Work out the finished part from the listing and answer in its coordinate system (mm). Round coordinates to 2 decimals unless told otherwise and drop trailing zeros. Write each loop counter-clockwise with the first axis right and the second up, starting at its lowest first coordinate (ties: lowest second). Pieces come first, ordered by that corner, then holes. Notation, with made-up numbers: M -15,15 L 41,15 A26 ccw 41,34 Z; hole C -14.5,18 d5. An arc over 180 degrees is marked long. Answer in a Markdown table with one row per item.
```python
from build123d import *

# Parameters (mm, degrees)
SKETCH1_W                  = 80
SKETCH1_H                  = 105
BOSS_EXTRUDE1_DEPTH        = 3
SKETCH2_R                  = 2.75
SKETCH2_R_2                = 25.05
CUT_EXTRUDE1_DEPTH         = 133.037873355
F_4_5_4_5_DIAMETER_HOLE1_D = 4.5
CHAMFER1_SIZE              = 2
M4_TAPPED_HOLE1_D          = 3.3
M4_TAPPED_HOLE1_DEPTH      = 10.1
M4_TAPPED_HOLE1_TIP        = 0.991420021


with BuildPart() as part:
    # Sketch1 → Boss-Extrude1 (new body)
    with BuildSketch(Plane.XY):
        with Locations((40, 52.5)):
            Rectangle(SKETCH1_W, SKETCH1_H)
    extrude(amount=BOSS_EXTRUDE1_DEPTH)

    # Sketch2 → Cut-Extrude1 (cut, through all)
    with BuildSketch(Plane.XY.offset(3)):
        with Locations((7.5, 97.5)):
            Circle(SKETCH2_R)
        with Locations((72.5, 97.5)):
            Circle(SKETCH2_R)
        with Locations((72.5, 7.5)):
            Circle(SKETCH2_R)
        with Locations((7.5, 7.5)):
            Circle(SKETCH2_R)
        with Locations((40, 65)):
            Circle(SKETCH2_R_2)
    extrude(amount=-CUT_EXTRUDE1_DEPTH, mode=Mode.SUBTRACT)

    # Ø4.5 (4.5) Diameter Hole1 (through all)
    with Locations(Plane.XY.offset(3)):
        with Locations((40, 95), (10, 65), (70, 65), (40, 35)):
            Hole(F_4_5_4_5_DIAMETER_HOLE1_D / 2)

    # Chamfer1
    chamfer1_edges = [part.edges().sort_by_distance(p)[0] for p in [
        (0, 105, 1.5),
        (80, 105, 1.5),
        (80, 0, 1.5),
        (0, 0, 1.5),
    ]]
    chamfer(chamfer1_edges, length=CHAMFER1_SIZE)

    # M4 Tapped Hole1
    with Locations(Plane.XY.offset(3)):
        with Locations((4, 87.5), (76, 87.5), (76, 22.5), (4, 22.5), (40, 65)):
            Hole(M4_TAPPED_HOLE1_D / 2, depth=M4_TAPPED_HOLE1_DEPTH)
            with Locations((0, 0, -(M4_TAPPED_HOLE1_DEPTH + M4_TAPPED_HOLE1_TIP / 2))):  # 118° drill point
                Cone(0, M4_TAPPED_HOLE1_D / 2, M4_TAPPED_HOLE1_TIP, mode=Mode.SUBTRACT)


solid = part.part
```
1. Given pin 1 (4 mm diameter, centred on x = 76, y = 22.5, fed in from -Z), flat-ended and moving along its own axis, determine where the tip first touches the part or whether it passes through.
Calculated:
| item | result |
|---|---|
| pin 1 | stops at z = 0 |
2. The part is cut by section C-C (y = 22.5). Determine the outline of the cut face in (x, z).
Calculated:
| item | result |
|---|---|
| outline | M 0,0 L 2.35,0 L 2.35,3 L 0,3 Z; M 5.65,0 L 74.35,0 L 74.35,3 L 5.65,3 Z; M 77.65,0 L 80,0 L 80,3 L 77.65,3 Z |
3. The part is cut by section D-D (z = 1.4). Count the separate pieces of the cut face and the enclosed holes in it, plus the area to 3 significant figures.
Calculated:
| item | result |
|---|---|
| separate pieces | 1 |
| enclosed holes | 13 |
| area | 6,230 mm² |
4. The part is cut by section B-B (x = 40). Determine the outline of the cut face in (y, z), plus the area to 3 significant figures.
Calculated:
| item | result |
|---|---|
| outline | M 0,0 L 32.75,0 L 32.75,3 L 0,3 Z; M 37.25,0 L 39.95,0 L 39.95,3 L 37.25,3 Z; M 90.05,0 L 92.75,0 L 92.75,3 L 90.05,3 Z; M 97.25,0 L 105,0 L 105,3 L 97.25,3 Z |
| area | 138 mm² |
5. Determine the mould class of faces 1 (the cylindrical face through (40.29, 37.23, 1.48)), 2 (the flat face through (1, 104, 1)), 3 (the flat face through (1, 1, 1)) for opening direction Y: released by +Y, released by -Y, zero draft, split by the parting line, or undercut.
Calculated:
| item | result |
|---|---|
| face 1 | undercut |
| face 2 | released by +Y |
| face 3 | released by -Y |
6. Consider line 1 along Y through (x, z) = (40, 1.35); line 2 along X through (y, z) = (97, 1.9); line 3 along Y through (x, z) = (8.5, 0.5). Determine where each line is inside the solid, lowest interval first. Write a range as from..to.
Calculated:
| item | result |
|---|---|
| line 1 | y = 0..32.75, 37.25..39.95, 90.05..92.75, 97.25..105 |
| line 2 | x = 0..4.8, 10.2..38.97, 41.03..69.8, 75.2..80 |
| line 3 | y = 0..4.94, 10.06..63.32, 66.68..94.94, 100.06..105 |
7. The part is cut by section A-A (y = 35). Determine the outline of the cut face in (x, z), plus the area to 4 significant figures.
Calculated:
| item | result |
|---|---|
| outline | M 0,0 L 37.75,0 L 37.75,3 L 0,3 Z; M 42.25,0 L 80,0 L 80,3 L 42.25,3 Z |
| area | 226.5 mm² |
